Source: CAD feature listing. Evaluate the final solid. Frame: model axes, mm. A direction names the side the tool comes from. Round coordinates to 2 decimals unless told otherwise and drop trailing zeros. Write each loop counter-clockwise with the first axis right and the second up, starting at its lowest first coordinate (ties: lowest second). Pieces come first, ordered by that corner, then holes. Notation, with made-up numbers: M 64.5,-22 L 72.5,-22 A19 ccw 72.5,-5 Z; hole C -22.75,25.25 d7. An arc over 180 degrees is marked long. Answer in a Markdown table with one row per item. Add a question column.
Item 1: Cut plane A-A on y = 0. Give the number of separate pieces and of enclosed holes in the cut face, and give its area (3 significant figures).
Item 2: Mould query, pull axis Y, two halves, no side actions, for faces 4 (the face through (20, 0, 1)), 5 (the face through (6.508, -2.008, -42.619)), 6 (the face through (10, 15, 1)), 7 (the face through (10, -7.08, 65)). Classes: released by +Y, released by -Y, zero draft, split by the parting line, or undercut.
Item 3: Cut plane B-B on z = -65. Return loops of the section in (x, y), and give its area (3 significant figures).
Item 4: Material intervals for probe 1 along Y at (x, z) = (15, -65); probe 2 along Y at (x, z) = (13, 66); probe 3 along Z at (x, y) = (10.25, 12.75), sorted ascending.
Item 5: Contact query for a flat-ended pin moving along its axis: pin 1 (5.5 mm diameter, centred on y = -1, z = -67.5, fed in from +X). Output: stop coordinate, or through.
Item 6: Set-up query: faces 1 (the face through (10, 0, 55)), 2 (the face through (16.648, 0.242, -34.505)), 3 (the face through (10, 0, 80)). Return all of +Z, -Z, +X, -X, +Y, -Y with unobstructed straight access to the full face (end or side cutting, diameter ignored); none if empty.
Item 7: Cut plane C-C on x = 15.5. Return loops of the section in (y, z).
from build123d import *

# Parameters (mm, degrees)
SKETCH_1_W                = 160
SKETCH_1_H                = 30
EXTRUDE_1_DEPTH           = 20
CUT_EXTRUDE_1_DEPTH       = 84.815273071
HOLE_WIZARD_1_D           = 6.6
HOLE_WIZARD_1_DEPTH       = 38
HOLE_WIZARD_1_CBORE_D     = 11
HOLE_WIZARD_1_CBORE_DEPTH = 6.8
HOLE_WIZARD_1_TIP         = 1.982840043
CHAMFER_1_SIZE            = 3


with BuildPart() as part:
    # 草图1 → 凸台-拉伸1 (new body)
    with BuildSketch(Plane(origin=(0, 0, 0), x_dir=(0, 0, -1), z_dir=(1, 0, 0))):
        Rectangle(SKETCH_1_W, SKETCH_1_H)
    extrude(amount=EXTRUDE_1_DEPTH)

    # 草图2 → 切除-拉伸1 (cut, through all)
    with BuildSketch(Plane(origin=(20, 0, 0), x_dir=(0, 0, -1), z_dir=(1, 0, 0))):
        with BuildLine():
            Line((-72.062216973, 7.079907586), (-57.937783027, 7.079907586))
            ThreePointArc((-57.937783027, 7.079907586), (-55, 0), (-57.937783027, -7.079907586))
            Line((-57.937783027, -7.079907586), (-72.062216973, -7.079907586))
            ThreePointArc((-72.062216973, -7.079907586), (-75, 0), (-72.062216973, 7.079907586))
        make_face()
    extrude(amount=-CUT_EXTRUDE_1_DEPTH, mode=Mode.SUBTRACT)

    # 打孔尺寸(%根据)内六角圆柱头螺钉的类型1
    with Locations(Plane(origin=(20, 0, 0), x_dir=(0, 0, -1), z_dir=(1, 0, 0))):
        with Locations((15, 0), (40, 0), (65, 0)):
            CounterBoreHole(HOLE_WIZARD_1_D / 2, HOLE_WIZARD_1_CBORE_D / 2, HOLE_WIZARD_1_CBORE_DEPTH, depth=HOLE_WIZARD_1_DEPTH)
            with Locations((0, 0, -(HOLE_WIZARD_1_DEPTH + HOLE_WIZARD_1_TIP / 2))):  # 118° drill point
                Cone(0, HOLE_WIZARD_1_D / 2, HOLE_WIZARD_1_TIP, mode=Mode.SUBTRACT)

    # 倒角1
    chamfer_1_edges = [part.edges().sort_by_distance(p)[0] for p in [
        (10, -15, -80),
        (10, -15, 80),
        (10, 15, 80),
        (10, 15, -80),
    ]]
    chamfer(chamfer_1_edges, length=CHAMFER_1_SIZE)


solid = part.part
Results below:
| question | item | result |
|---|---|---|
| 1 | separate pieces | 5 |
| 1 | enclosed holes | 0 |
| 1 | area | 2,310 mm2 |
| 2 | face 4 | zero draft |
| 2 | face 5 | undercut |
| 2 | face 6 | released by +Y |
| 2 | face 7 | undercut |
| 3 | outline | M 0,-15 L 20,-15 L 20,-5.5 L 13.2,-5.5 L 13.2,-3.3 L 0,-3.3 Z; M 0,3.3 L 13.2,3.3 L 13.2,5.5 L 20,5.5 L 20,15 L 0,15 Z |
| 3 | area | 438 mm2 |
| 4 | probe 1 | -15 to -5.5, 5.5 to 15 |
| 4 | probe 2 | -15 to -7.08, 7.08 to 15 |
| 4 | probe 3 | -79.25 to 79.25 |
| 5 | pin 1 | x = 13.2 |
| 6 | face 1 | +X, -X |
| 6 | face 2 | +X |
| 6 | face 3 | +Z, +X, -X, +Y, -Y |
| 7 | outline | M -15,-77 L -12,-80 L 12,-80 L 15,-77 L 15,77 L 12,80 L -12,80 L -15,77 Z; hole M -7.08,57.94 A10 ccw 7.08,57.94 L 7.08,72.06 A10 ccw -7.08,72.06 Z; hole C 0,-65 d11; hole C 0,-40 d11; hole C 0,-15 d11 |
